from build123d import *

# Parameters (mm, degrees)
SKETCH1_R           = 5
BOSS_EXTRUDE1_DEPTH = 10


with BuildPart() as part:
    # Sketch1 → Boss-Extrude1 (new body)
    with BuildSketch(Plane.XY):
        with BuildLine():
            Line((5, 0), (95, 0))
            ThreePointArc((95, 0), (98.535533906, -1.464466094), (100, -5))
            Line((100, -5), (100, -115))
            ThreePointArc((100, -115), (98.535533906, -118.535533906), (95, -120))
            Line((95, -120), (5, -120))
            ThreePointArc((5, -120), (1.464466094, -118.535533906), (0, -115))
            Line((0, -115), (0, -5))
            ThreePointArc((0, -5), (1.464466094, -1.464466094), (5, 0))
        make_face()
        with Locations((12.5, -17.5)):
            Circle(SKETCH1_R, mode=Mode.SUBTRACT)
        with Locations((87.5, -17.5)):
            Circle(SKETCH1_R, mode=Mode.SUBTRACT)
        with Locations((87.5, -102.5)):
            Circle(SKETCH1_R, mode=Mode.SUBTRACT)
        with Locations((12.5, -102.5)):
            Circle(SKETCH1_R, mode=Mode.SUBTRACT)
    extrude(amount=BOSS_EXTRUDE1_DEPTH)


solid = part.part
Read the model definition and answer for the solid it produces. Units are mm, in the model's axes. Round coordinates to 2 decimals unless told otherwise and drop trailing zeros. Write each loop counter-clockwise with the first axis right and the second up, starting at its lowest first coordinate (ties: lowest second). Pieces come first, ordered by that corner, then holes.
Q1. A flat-ended cylindrical pin translates along its axis: P1, Ø8, axis at x = 87.5, y = -17.5, coming from the +Z side. Find the tip coordinate at first contact, or state that the pin passes through.
Values:
P1: passes through
Q2. The mould has two halves that part along Y. Classify faces 1 (the face through (14.807, -21.936, 4.93)), 2 (the face through (1, -2, 5)), 3 (the face through (100, -59, 5)), 4 (the face through (51, -120, 5)): released by +Y, released by -Y, zero draft, split by the parting line, or undercut.
Values:
face 1: undercut
face 2: released by +Y
face 3: zero draft
face 4: released by -Y
Q3. Straight lines are drawn through the part: line 1 (Y direction, x = 87.5, z = 8); line 2 (Y direction, x = 85, z = 7.25); line 3 (X direction, y = -104, z = 7). For each, find the intervals that lie inside material, in ascending order.
Values:
line 1: y = -120 to -107.5, -97.5 to -22.5, -12.5 to 0
line 2: y = -120 to -106.83, -98.17 to -21.83, -13.17 to 0
line 3: x = 0 to 7.73, 17.27 to 82.73, 92.27 to 100
Q4. Find section C-C on y = -102.5. Determine the outline of the cut face in (x, z).
Values:
outline: (0, 0) - (7.5, 0) - (7.5, 10) - (0, 10) - close; (17.5, 0) - (82.5, 0) - (82.5, 10) - (17.5, 10) - close; (92.5, 0) - (100, 0) - (100, 10) - (92.5, 10) - close
Q5. Find section B-B on x = 12.5. Determine the outline of the cut face in (y, z), and give its area (3 significant figures).
Values:
outline: (-120, 0) - (-107.5, 0) - (-107.5, 10) - (-120, 10) - close; (-97.5, 0) - (-22.5, 0) - (-22.5, 10) - (-97.5, 10) - close; (-12.5, 0) - (0, 0) - (0, 10) - (-12.5, 10) - close
area: 1,000 mm2
Q6. Find section A-A on z = 5.5. Determine the outline of the cut face in (x, y).
Values:
outline: (0, -115) arc R5 ccw to (5, -120) - (95, -120) arc R5 ccw to (100, -115) - (100, -5) arc R5 ccw to (95, 0) - (5, 0) arc R5 ccw to (0, -5) - close; hole circle Ø10 at (12.5, -102.5); hole circle Ø10 at (12.5, -17.5); hole circle Ø10 at (87.5, -102.5); hole circle Ø10 at (87.5, -17.5)
